Geometry: final body of the model. Coordinates: model frame, mm. Face numbers are marked on the shaded views. A direction names the side the tool comes from. Give positions to 0.01 mm unless a question says otherwise; leave off trailing zeros. Write each loop counter-clockwise with the first axis right and the second up, starting at its lowest first coordinate (ties: lowest second). Pieces come first, ordered by that corner, then holes.
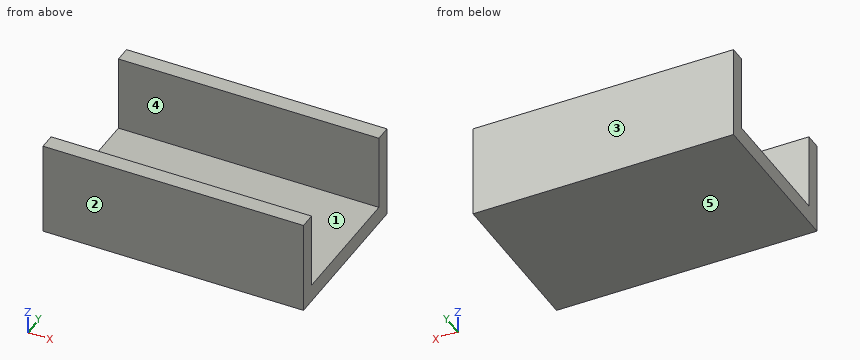
```python
from build123d import *

# Parameters (mm, degrees)
SKETCH1_W           = 80
SKETCH1_H           = 50
BOSS_EXTRUDE1_DEPTH = 28.83
SKETCH2_W           = 23.467762578
SKETCH2_H           = 40.294008895
CUT_EXTRUDE1_DEPTH  = 99.646687223


with BuildPart() as part:
    # Sketch1 → Boss-Extrude1 (new body)
    with BuildSketch(Plane.XY):
        with Locations((40, 25)):
            Rectangle(SKETCH1_W, SKETCH1_H)
    extrude(amount=BOSS_EXTRUDE1_DEPTH)

    # Sketch2 → Cut-Extrude1 (cut, through all)
    with BuildSketch(Plane(origin=(80, 0, 0), x_dir=(0, 0, -1), z_dir=(1, 0, 0))):
        with Locations((-17.096118711, 25.002275375)):
            Rectangle(SKETCH2_W, SKETCH2_H)
    extrude(amount=-CUT_EXTRUDE1_DEPTH, mode=Mode.SUBTRACT)


solid = part.part
```
Item 1: Pin query (flat end, axial travel): pin 1 Ø4 at (x, y) = (44.5, 18.5) entering from +Z. Return the tip coordinate at first contact, or that it passes through.
Found:
pin 1: stops at z = 5.36
Item 2: Pull-direction query (Y, two-part tool) for the marked faces 1, 2 and 3; classes: +Y half, -Y half, draft (parallel to the pull), parting line (faces both ways), or undercut.
Found:
face 1: undercut
face 2: -Y half
face 3: +Y half
Item 3: Line query: L1, parallel to Y at x = 6, z = 22.75; L2, parallel to Z at x = 30.5, y = 41. Output: solid intervals per line, ascending.
Found:
L1: y = 0 to 4.86, 45.15 to 50
L2: z = 0 to 5.36
Item 4: Section C-C, the plane y = 37. Return the cut outline in (x, z), plus the area to 3 significant figures.
Found:
outline: (0, 0) - (80, 0) - (80, 5.36) - (0, 5.36) - close
area: 429 mm2
Item 5: Section B-B, the plane x = 14.5. Return the cut outline in (y, z).
Found:
outline: (0, 0) - (50, 0) - (50, 28.83) - (45.15, 28.83) - (45.15, 5.36) - (4.86, 5.36) - (4.86, 28.83) - (0, 28.83) - close
Item 6: Reachability of the marked faces 4 and 5 from +Z, -Z, +X, -X, +Y, -Y: full face, straight path, thin tool, end or side. Return the list, or none.
Found:
face 4: +Z, +X, -X
face 5: -Z, +X, -X, +Y, -Y
Item 7: Section A-A, the plane z = 18.25. Return the cut outline in (x, y), plus the area to 3 significant figures.
Found:
outline: (0, 0) - (80, 0) - (80, 4.86) - (0, 4.86) - close; (0, 45.15) - (80, 45.15) - (80, 50) - (0, 50) - close
area: 776 mm2
